For this review, use the dimensioned drawing (mm, ordinates from the lowest corner) and the shaded views. A direction names the side the tool comes from. Round coordinates to 2 decimals unless told otherwise and drop trailing zeros. Loops run counter-clockwise (first coordinate to the right, second up) from the corner with the lowest first, then second, coordinate; pieces in that order, holes last. Notation, with made-up numbers: (25.5, 27.25) -> (50.5, 27.25) arc R12 ccw to (50.5, 45.25) -> close; hole circle Ø10 at (59.5, 53). An arc over 180 degrees is marked (long way). Answer as CSV lines item,"result". Start each with the question number.
(1) To check wall thickness, follow line 1 (X direction, y = 16.5, z = 2.9); line 2 (X direction, y = 19.5, z = 4.65); line 3 (Z direction, x = 0.75, y = 10.75). State the ranges of each line that lie inside material, in increasing order. Write a range as from..to.
(2) Take a section at B-B, the plane x = 3. Write out the cut boundary in (y, z) (3 decimals).
(3) Take a section at A-A, the plane z = 3. Write out the cut boundary in (x, y) (3 decimals).
(4) For P1, Ø3, axis at y = 16, z = 2.5, coming from the +X side (3 decimals); P2, Ø1.5, axis at y = 7.5, z = 4.5, coming from the +X side, all flat-tipped, find the tip position at first contact; note any pin that passes through.
(5) Take a section at C-C, the plane y = 4.25. Write out the cut boundary in (x, z), and give its area (3 significant figures).
(6) Machinability: for the marked faces 1 and 2, which of the approach directions +Z, -Z, +X, -X, +Y, -Y give a long, thin tool a straight path to every point of the face, cutting with its end or side? Answer none if there is none.
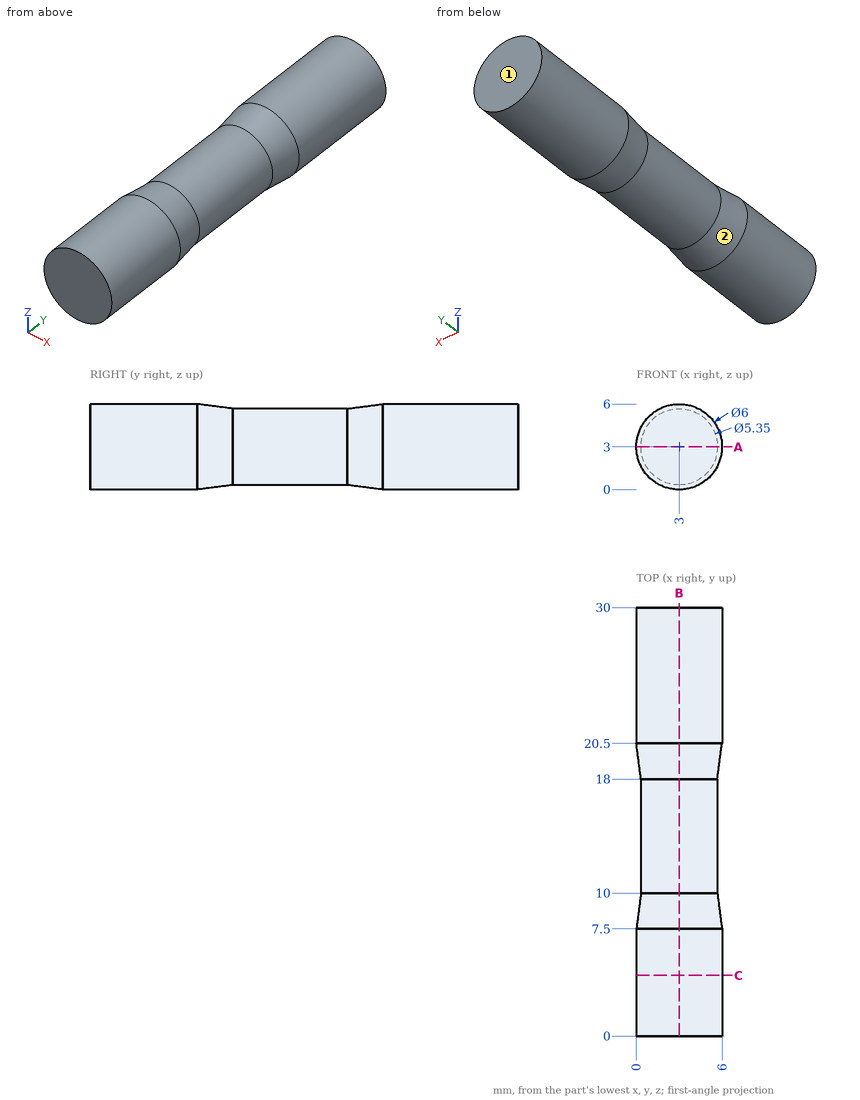
The answers:
1,line 1,"0.33..5.67"
1,line 2,"0.65..5.35"
1,line 3,"1.55..4.45"
2,outline,"(0, 0) -> (7.5, 0) -> (10, 0.325) -> (18, 0.325) -> (20.5, 0) -> (30, 0) -> (30, 6) -> (20.5, 6) -> (18, 5.675) -> (10, 5.675) -> (7.5, 6) -> (0, 6) -> close"
3,outline,"(0, 0) -> (6, 0) -> (6, 7.5) -> (5.675, 10) -> (5.675, 18) -> (6, 20.5) -> (6, 30) -> (0, 30) -> (0, 20.5) -> (0.325, 18) -> (0.325, 10) -> (0, 7.5) -> close"
4,P1,"x = 5.675"
4,P2,"x = 5.9"
5,outline,"circle Ø6 at (3, 3)"
5,area,"28.3 mm²"
6,face 1,"+Z, -Z, +X, -X, +Y"
6,face 2,"none"
